Geometry check sheet. Reference: drawing and pictorial views, mm from the part's lowest x, y, z. A direction names the side the tool comes from. Round coordinates to 2 decimals unless told otherwise and drop trailing zeros. Write each loop counter-clockwise with the first axis right and the second up, starting at its lowest first coordinate (ties: lowest second). Pieces come first, ordered by that corner, then holes. Notation, with made-up numbers: M 48.25,-4 L 52.25,-4 A8 ccw 52.25,4 Z; hole C 71,63 d8. An arc over 180 degrees is marked long. One line per question, with ' | ' between items.
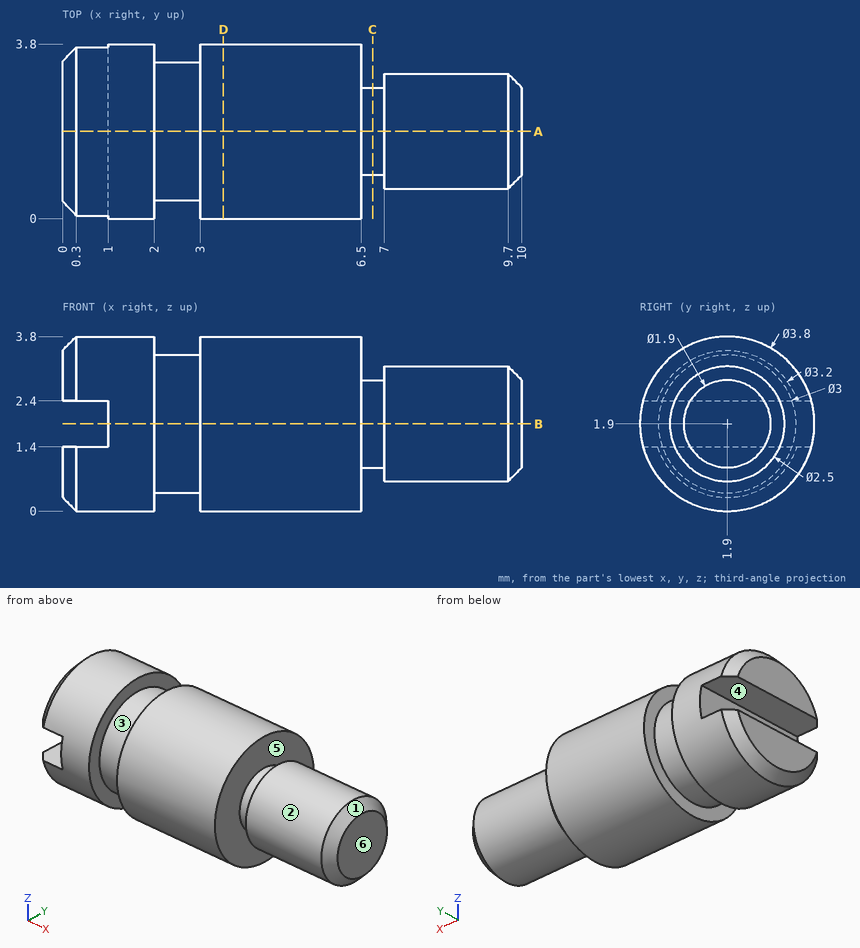
1. Mould release check, pull along X, two halves, no side actions. Record for the marked faces 1, 2 and 3: pulls with the +X half, pulls with the -X half, needs draft (parallel to the pull), parting line crosses it, or undercut.
Results:
face 1: pulls with the +X half | face 2: needs draft | face 3: undercut
2. Section check A-A, the plane y = 1.9. Record the cut outline in (x, z).
Results:
outline: M 0,0.3 L 0.3,0 L 2,0 L 2,0.4 L 3,0.4 L 3,0 L 6.5,0 L 6.5,0.95 L 7,0.95 L 7,0.65 L 9.7,0.65 L 10,0.95 L 10,2.85 L 9.7,3.15 L 7,3.15 L 7,2.85 L 6.5,2.85 L 6.5,3.8 L 3,3.8 L 3,3.4 L 2,3.4 L 2,3.8 L 0.3,3.8 L 0,3.5 L 0,2.4 L 1,2.4 L 1,1.4 L 0,1.4 Z
3. Section check D-D, the plane x = 3.5. Record the cut outline in (y, z), then the cut area to 3 significant figures.
Results:
outline: C 1.9,1.9 d3.8 | area: 11.3 mm2
4. Tool access check on the marked faces 4, 5 and 6. Record the directions out of +Z, -Z, +X, -X, +Y, -Y that give a thin tool (end or side, any length) a straight path to the whole face; none if there is none.
Results:
face 4: -X, +Y, -Y | face 5: none | face 6: +Z, -Z, +X, +Y, -Y
5. Section check C-C, the plane x = 6.75. Record the cut outline in (y, z).
Results:
outline: C 1.9,1.9 d1.9
6. Go/stop test with flat-tipped pins: P1, Ø0.5, axis at y = 2.5, z = 2, coming from the -X side; P2, Ø1.5, axis at x = 7, z = 1, coming from the +Y side. Record where each tip stops, or that it passes through.
Results:
P1: stops at x = 1 | P2: stops at y = 3.77
7. Thickness scan on line 1 (X direction, y = 2.95, z = 3.2); line 2 (Y direction, x = 9.75, z = 1.05); line 3 (Z direction, x = 4.25, y = 0.25). Record the ranges inside material, lowest first.
Results:
line 1: x = 0.07 to 2, 3 to 6.5 | line 2: y = 1.05 to 2.75 | line 3: z = 0.96 to 2.84
8. Section check B-B, the plane z = 1.9. Record the cut outline in (x, y).
Results:
outline: M 1,0 L 2,0 L 2,0.4 L 3,0.4 L 3,0 L 6.5,0 L 6.5,0.95 L 7,0.95 L 7,0.65 L 9.7,0.65 L 10,0.95 L 10,2.85 L 9.7,3.15 L 7,3.15 L 7,2.85 L 6.5,2.85 L 6.5,3.8 L 3,3.8 L 3,3.4 L 2,3.4 L 2,3.8 L 1,3.8 Z
